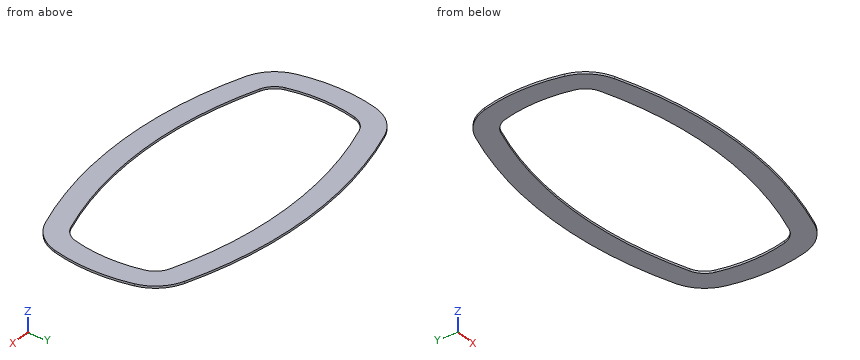
```python
from build123d import *

# Parameters (mm, degrees)
BOSS_EXTRUDE1_DEPTH = 3


with BuildPart() as part:
    # Sketch1 → Boss-Extrude1 (new body)
    with BuildSketch(Plane.XY):
        with BuildLine():
            ThreePointArc((-185.063461818, 97.930029155), (0, 130), (185.063461818, 97.930029155))
            ThreePointArc((185.063461818, 97.930029155), (209.308091137, 81.748238793), (223.065798362, 56.050420168))
            ThreePointArc((223.065798362, 56.050420168), (230, 0), (223.065798362, -56.050420168))
            ThreePointArc((223.065798362, -56.050420168), (209.308091137, -81.748238793), (185.063461818, -97.930029155))
            ThreePointArc((185.063461818, -97.930029155), (0, -130), (-185.063461818, -97.930029155))
            ThreePointArc((-185.063461818, -97.930029155), (-209.308091137, -81.748238793), (-223.065798362, -56.050420168))
            ThreePointArc((-223.065798362, -56.050420168), (-230, 0), (-223.065798362, 56.050420168))
            ThreePointArc((-223.065798362, 56.050420168), (-209.308091137, 81.748238793), (-185.063461818, 97.930029155))
        make_face()
        with BuildLine():
            ThreePointArc((-174.969091173, 69.679300292), (0, 100), (174.969091173, 69.679300292))
            ThreePointArc((174.969091173, 69.679300292), (187.091405833, 61.588405111), (193.970259445, 48.739495798))
            ThreePointArc((193.970259445, 48.739495798), (200, 0), (193.970259445, -48.739495798))
            ThreePointArc((193.970259445, -48.739495798), (187.091405833, -61.588405111), (174.969091173, -69.679300292))
            ThreePointArc((174.969091173, -69.679300292), (0, -100), (-174.969091173, -69.679300292))
            ThreePointArc((-174.969091173, -69.679300292), (-187.091405833, -61.588405111), (-193.970259445, -48.739495798))
            ThreePointArc((-193.970259445, -48.739495798), (-200, 0), (-193.970259445, 48.739495798))
            ThreePointArc((-193.970259445, 48.739495798), (-187.091405833, 61.588405111), (-174.969091173, 69.679300292))
        make_face(mode=Mode.SUBTRACT)
    extrude(amount=BOSS_EXTRUDE1_DEPTH)


solid = part.part
```
Model file for the job. Use its own axes, mm. Coordinates: 2 decimals unless noted, no trailing zeros. Loops run counter-clockwise (first coordinate to the right, second up) from the corner with the lowest first, then second, coordinate; pieces in that order, holes last. Notation, with made-up numbers: M -1,-33.75 L 35,-33.75 A23 ccw 35,-19.75 Z; hole C 13.25,69.5 d6. An arc over 180 degrees is marked long. Use CSV: the item, a comma, the result in double quotes. Start each with the question number.
1. Band-saw the part on A-A, the plane z = 1.3. List the corners of the cut face in (x, y).
2. Band-saw the part on B-B, the plane x = 164. List the corners of the cut face in (y, z).
3. Flat gauge pins, fed straight in: pin 1 (1 mm diameter, centred on y = 64, z = 1.5, fed in from -X); pin 2 (1.5 mm diameter, centred on y = -71.5, z = 1.5, fed in from +X). Where does each tip first touch, or does it go through?
4. Probe probe 1 along X at (y, z) = (-27, 2.5); probe 2 along X at (y, z) = (-25, 0.25); probe 3 along Y at (x, z) = (67, 2.1). List the from-to ranges inside material, lowest first. Write a range as [from, to].
5. Band-saw the part on C-C, the plane y = 18.5. List the corners of the cut face in (x, z).
Entries:
1,outline,"M -223.07,-56.05 A60 ccw -185.06,-97.93 A550 ccw 185.06,-97.93 A60 ccw 223.07,-56.05 A230 ccw 223.07,56.05 A60 ccw 185.06,97.93 A550 ccw -185.06,97.93 A60 ccw -223.07,56.05 A230 ccw Z; hole M -193.97,-48.74 A30 ccw -174.97,-69.68 A520 ccw 174.97,-69.68 A30 ccw 193.97,-48.74 A200 ccw 193.97,48.74 A30 ccw 174.97,69.68 A520 ccw -174.97,69.68 A30 ccw -193.97,48.74 A200 ccw Z"
2,outline,"M -104.98,0 L -73.46,0 L -73.46,3 L -104.98,3 Z; M 73.46,0 L 104.98,0 L 104.98,3 L 73.46,3 Z"
3,pin 1,"stops at x = -220.67"
3,pin 2,"stops at x = 217.22"
4,probe 1,"x = [-228.41, -198.17], [198.17, 228.41]"
4,probe 2,"x = [-228.64, -198.43], [198.43, 228.64]"
4,probe 3,"y = [-125.9, -95.67], [95.67, 125.9]"
5,outline,"M -229.25,0 L -199.14,0 L -199.14,3 L -229.25,3 Z; M 199.14,0 L 229.25,0 L 229.25,3 L 199.14,3 Z"
